Design review of the part shown in the three views and the two pictorial views. Dimensions are in mm from the part's minimum x, y and z. A direction names the side the tool comes from. Round coordinates to 2 decimals unless told otherwise and drop trailing zeros. Order: outer loops, then holes, each group sorted by start corner. A loop starts at its lowest first (then second) coordinate and runs counter-clockwise, first axis right, second up.
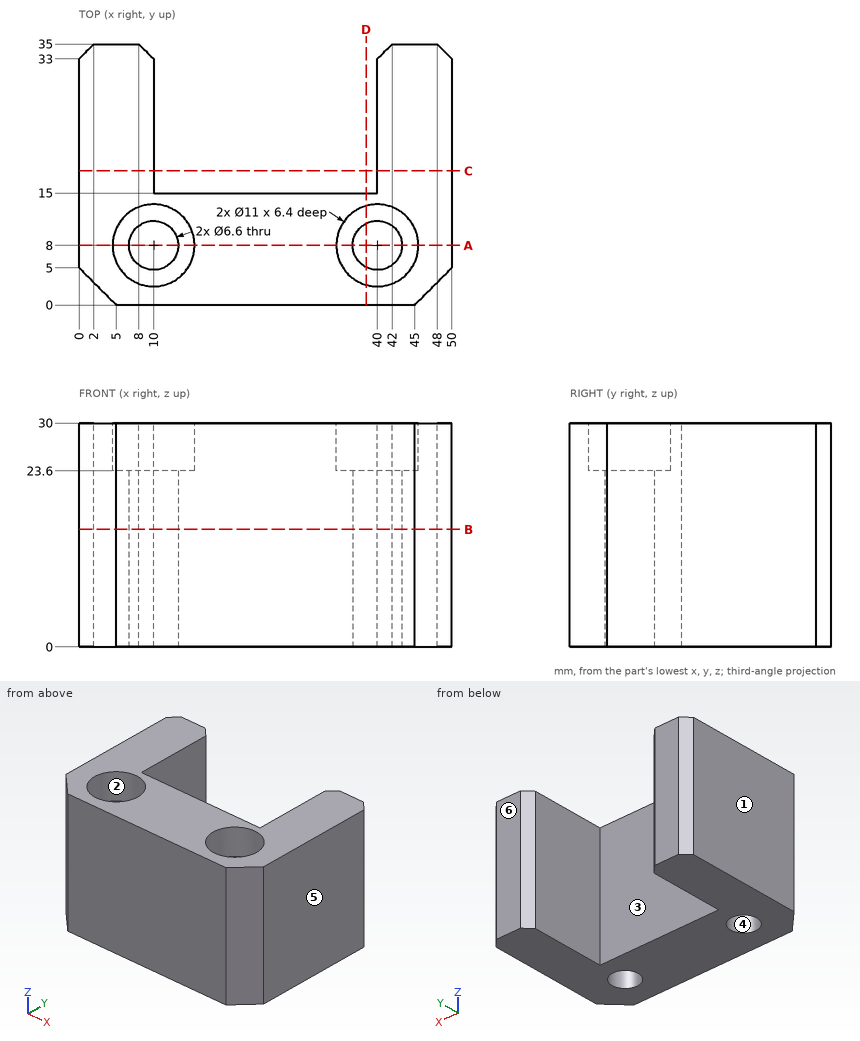
(1) Add section C-C on y = 18. Give the boundary of the cut face in (x, z), plus the area to 3 significant figures.
(2) Add section B-B on z = 15.75. Give the boundary of the cut face in (x, y).
(3) Wall thickness on L1, parallel to X at y = 7, z = 24; L2, parallel to X at y = 10, z = 5; L3, parallel to X at y = 27, z = 15.25: over which ranges is each line inside the solid? List them lowest first.
(4) Clearance check with flat-ended pins moving along their axes: P1, Ø4, axis at x = 40, y = 8, coming from the -Z side; P2, Ø5.5, axis at x = 40.5, y = 6, coming from the +Z side. State where each tip first meets the part, or that it passes through.
(5) Add section D-D on x = 38.5. Give the boundary of the cut face in (y, z), plus the area to 3 significant figures.
(6) Tool access review of the marked faces 1, 2 and 3: name each direction out of +Z, -Z, +X, -X, +Y, -Y from which nothing blocks a thin tool from reaching the whole face with its end or side.
(7) Add section A-A on y = 8. Give the boundary of the cut face in (x, z), plus the area to 3 significant figures.
(8) Draft analysis for pull direction Y (two halves, no side actions). For the marked faces 4, 5 and 6, state which applies: pulls with the +Y half, pulls with the -Y half, needs draft (parallel to the pull), parting line crosses it, or undercut.
Here are the results:
1. outline: (0, 0) - (10, 0) - (10, 30) - (0, 30) - close; (40, 0) - (50, 0) - (50, 30) - (40, 30) - close
1. area: 600 mm2
2. outline: (0, 5) - (5, 0) - (45, 0) - (50, 5) - (50, 33) - (48, 35) - (42, 35) - (40, 33) - (40, 15) - (10, 15) - (10, 33) - (8, 35) - (2, 35) - (0, 33) - close; hole circle Ø6.6 at (10, 8); hole circle Ø6.6 at (40, 8)
3. L1: x = 0 to 4.59, 15.41 to 34.59, 45.41 to 50
3. L2: x = 0 to 7.38, 12.62 to 37.38, 42.62 to 50
3. L3: x = 0 to 10, 40 to 50
4. P1: passes through
4. P2: stops at z = 23.6
5. outline: (0, 0) - (5.06, 0) - (5.06, 23.6) - (2.71, 23.6) - (2.71, 30) - (0, 30) - close; (10.94, 0) - (15, 0) - (15, 30) - (13.29, 30) - (13.29, 23.6) - (10.94, 23.6) - close
5. area: 244 mm2
6. face 1: +Z, -Z, -X, +Y, -Y
6. face 2: +Z
6. face 3: +Z, -Z, +Y
7. outline: (0, 0) - (6.7, 0) - (6.7, 23.6) - (4.5, 23.6) - (4.5, 30) - (0, 30) - close; (13.3, 0) - (36.7, 0) - (36.7, 23.6) - (34.5, 23.6) - (34.5, 30) - (15.5, 30) - (15.5, 23.6) - (13.3, 23.6) - close; (43.3, 0) - (50, 0) - (50, 30) - (45.5, 30) - (45.5, 23.6) - (43.3, 23.6) - close
7. area: 1,050 mm2
8. face 4: undercut
8. face 5: needs draft
8. face 6: pulls with the +Y half
